from build123d import *

# Parameters (mm, degrees)
EXTRUDE_1_DEPTH          = 25
SKETCH_3_W               = 68.112999437
SKETCH_3_H               = 98.020483962
CUT_EXTRUDE_1_DEPTH      = 16
SKETCH_4_R               = 6.5
CUT_EXTRUDE_2_DEPTH      = 117.308950023
FILLET_1_R               = 3
HOLE_WIZARD_1_AT_2_COUNT = 2
HOLE_WIZARD_1_AT_2_PITCH = 50.998600142
FILLET_2_R               = 3


with BuildPart() as part:
    # 草图2 → 凸台-拉伸1 (new, symmetric)
    with BuildSketch(Plane.XY):
        with BuildLine():
            Line((0, 0), (0, 80))
            Line((0, 80), (9.710190579, 80))
            ThreePointArc((9.710190579, 80), (14.919635909, 79.54423259), (19.970794879, 78.190778624))
            Line((19.970794879, 78.190778624), (46.296148462, 68.609133513))
            ThreePointArc((46.296148462, 68.609133513), (67.815421572, 33.834375668), (39.025067596, 4.791675789))
            Line((39.025067596, 4.791675789), (0, 0))
        make_face()
    extrude(amount=EXTRUDE_1_DEPTH, both=True)

    # 草图3 → 切除-拉伸1 (cut, symmetric)
    with BuildSketch(Plane.XY):
        with Locations((44.056499718, 41.123691615)):
            Rectangle(SKETCH_3_W, SKETCH_3_H)
    extrude(amount=CUT_EXTRUDE_1_DEPTH, both=True, mode=Mode.SUBTRACT)

    # 草图4 → 切除-拉伸2 (cut, through all)
    with BuildSketch(Plane.XY.offset(25)):
        with Locations((35, 37.573220687)):
            Circle(SKETCH_4_R)
    extrude(amount=-CUT_EXTRUDE_2_DEPTH, mode=Mode.SUBTRACT)

    # 圆角1
    fillet_1_edges = [part.edges().sort_by_distance(p)[0] for p in [
        (33.13347167, 73.399956068, 25),
        (14.919635909, 79.54423259, 25),
        (4.855095289, 80, 25),
        (19.512533798, 2.395837894, 25),
        (4.855095289, 80, -25),
        (14.919635909, 79.54423259, -25),
        (67.815421572, 33.834375668, 25),
        (33.13347167, 73.399956068, -25),
        (67.815421572, 33.834375668, -25),
        (19.512533798, 2.395837894, -25),
    ]]
    fillet(fillet_1_edges, radius=FILLET_1_R)

    # 草图6 → 打孔尺寸(%根据)内六角花形半沉头螺钉的类型1 (revolve, cut)
    with BuildSketch(Plane(origin=(10, 65.998600142, 0), x_dir=(0, 0, -1), z_dir=(0, 1, 0))):
        Polygon((0, 0), (0, 10), (5.5, 10), (5.5, 4.65), (10.15, 0), align=None)
    hole_wizard_1 = revolve(axis=Axis((16.35, 65.998600142, 0), (-1, 0, 0)), mode=Mode.SUBTRACT)

    # 打孔尺寸(%根据)内六角花形半沉头螺钉的类型1 at 2: 打孔尺寸(%根据)内六角花形半沉头螺钉的类型1 ×2
    with Locations(*[(0, -i * HOLE_WIZARD_1_AT_2_PITCH, 0) for i in range(1, HOLE_WIZARD_1_AT_2_COUNT)]):
        add(hole_wizard_1, mode=Mode.SUBTRACT)

    # 圆角2
    fillet_2_edges = [part.edges().sort_by_distance(p)[0] for p in [
        (10, 40.613222876, -16),
        (10, 40.613222876, 16),
    ]]
    fillet(fillet_2_edges, radius=FILLET_2_R)


solid = part.part
Here's how the part is built. I have some questions about the finished solid (model axes, mm). A direction names the side the tool comes from. Coordinates: 2 decimals unless noted, no trailing zeros. Order: outer loops, then holes, each group sorted by start corner. A loop starts at its lowest first (then second) coordinate and runs counter-clockwise, first axis right, second up. Notation, with made-up numbers: (44, 84) -> (101, 84) arc R14 ccw to (101, 89) -> close; hole circle Ø3 at (17, 22). An arc over 180 degrees is marked (long way). Answer in a Markdown table with one row per item.
(1) On a 3-axis mill with a long thin cutter (end or side, diameter ignored), from which of +Z, -Z, +X, -X, +Y, -Y can I reach the whole of each face in a straight line? I mean faces 5 (the face through (10.9, 41.16, -15.14)), 6 (the face through (14.513, 79.613, 16.399)). Say none if no direction works.
Answer key:
| item | result |
|---|---|
| face 5 | +X, +Y, -Y |
| face 6 | +Z, -Z, +X, +Y |
(2) Will these pins go through, and if not, where does the flat tip stop? pin 1 Ø2 at (y, z) = (64, -7) entering from +X; pin 2 Ø2 at (x, z) = (40.5, -16.5) entering from +Y; pin 3 Ø4 at (x, z) = (53.5, -17.5) entering from +Y; pin 4 Ø17 at (x, y) = (35, 37.57) entering from -Z.
Answer key:
| item | result |
|---|---|
| pin 1 | x = 8.13 |
| pin 2 | y = 71.08 |
| pin 3 | y = 66.18 |
| pin 4 | z = -25 |
(3) Thinking about a two-plate mould opening in Y: for faces 1 (the face through (4.92, 79.1, -24.14)), 2 (the face through (2.71, 20.37, 1.19)), 3 (the face through (5.641, 69.522, 4.595)), 4 (the face through (67.88, 34.45, -18.96)), which applies, +Y half, -Y half, draft (parallel to the pull), parting line (faces both ways), or undercut?
Answer key:
| item | result |
|---|---|
| face 1 | +Y half |
| face 2 | undercut |
| face 3 | undercut |
| face 4 | parting line |
(4) I want a section at B-B on y = 35. Count the separate pieces of the cut face and the enclosed holes in it, then the cut area to 3 significant figures.
Answer key:
| item | result |
|---|---|
| separate pieces | 3 |
| enclosed holes | 0 |
| area | 1,330 mm^2 |
(5) Please list where these lines run through material, in increasing order: probe 1 along Z at (x, y) = (44, 36); probe 2 along Y at (x, z) = (3.5, 0); probe 3 along Z at (x, y) = (11.5, 33.5).
Answer key:
| item | result |
|---|---|
| probe 1 | -25 to -16, 16 to 25 |
| probe 2 | 0.43 to 9.5, 20.5 to 60.5, 71.5 to 80 |
| probe 3 | -25 to -15.6, 15.6 to 25 |
(6) I want a section at A-A on z = 0. List the corners of the cut face in (x, y) for me, then the cut area to 3 significant figures.
Answer key:
| item | result |
|---|---|
| outline | (0, 0) -> (10, 1.23) -> (10, 4.85) -> (5.35, 9.5) -> (0, 9.5) -> close; (0, 20.5) -> (5.35, 20.5) -> (10, 25.15) -> (10, 55.85) -> (5.35, 60.5) -> (0, 60.5) -> close; (0, 71.5) -> (5.35, 71.5) -> (10, 76.15) -> (10, 80) arc R30 ccw to (9.71, 80) -> (0, 80) -> close |
| area | 531 mm^2 |
